```python
from build123d import *

# Parameters (mm, degrees)
BASE_EXTRUDE_DEPTH      = 1.5
BASE_EXTRUDE_DEPTH_BACK = 1.5
SKETCH1_R               = 2


with BuildPart() as part:
    # Sketch1 → Base-Extrude (new, two sides: drawn at the far end of the back side and taken through both)
    with BuildSketch(Plane.XY.offset(-BASE_EXTRUDE_DEPTH_BACK)):
        with BuildLine():
            Line((-14.708808387, -54.894020219), (-16.435009364, -61.336289969))
            ThreePointArc((-16.435009364, -61.336289969), (0, 63.5), (16.435009364, -61.336289969))
            Line((16.435009364, -61.336289969), (14.708808387, -54.894020219))
            ThreePointArc((14.708808387, -54.894020219), (17.560433321, -49.007812256), (23.796756449, -50.979482305))
            ThreePointArc((23.796756449, -50.979482305), (25.28518113, -52.085758206), (27.1261898, -51.862282302))
            ThreePointArc((27.1261898, -51.862282302), (0, 54.2), (-27.1261898, -51.862282302))
            ThreePointArc((-27.1261898, -51.862282302), (-25.28518113, -52.085758206), (-23.796756449, -50.979482305))
            ThreePointArc((-23.796756449, -50.979482305), (-17.560433321, -49.007812256), (-14.708808387, -54.894020219))
        make_face()
        with Locations((-19.733291854, -54.327131275)):
            Circle(SKETCH1_R, mode=Mode.SUBTRACT)
        with Locations(Location((19.733291854, -54.327131275, 0), (0, 0, 180))):
            Circle(SKETCH1_R, mode=Mode.SUBTRACT)
    extrude(amount=BASE_EXTRUDE_DEPTH + BASE_EXTRUDE_DEPTH_BACK)


solid = part.part
```
Source: CAD feature listing. Evaluate the final solid. Frame: model axes, mm. A direction names the side the tool comes from. Coordinates: 2 decimals unless noted, no trailing zeros. Order: outer loops, then holes, each group sorted by start corner. A loop starts at its lowest first (then second) coordinate and runs counter-clockwise, first axis right, second up. Notation, with made-up numbers: M -29.5,68.25 L -10.5,68.25 A22 cw -10.5,87.25 Z; hole C -12.75,81.5 d3. An arc over 180 degrees is marked long. Write each question's results on one line, items separated by ' | '. Start each with the question number.
1) Section query D-D (x = 0). Return the cut outline in (y, z), plus the area to 3 significant figures.
2) Section query C-C (x = -40). Return the cut outline in (y, z).
3) Section query B-B (z = -0.95). Return the cut outline in (x, y) (3 decimals).
4) Contact query for flat-ended pins moving along their axis: pin 1 Ø1.5 at (x, z) = (-36.5, 1) entering from -Y; pin 2 Ø1.5 at (y, z) = (-0.5, 0) entering from +X; pin 3 Ø5 at (x, y) = (19.73, -54.33) entering from +Z. Output: stop coordinate, or through.
5) Draft query along Y for faces 4 (the face through (-15.56, -58.07, -0.02)), 5 (the face through (-25.311, -52.092, -0.021)), 6 (the face through (-2.56, 63.45, -0.02)). Return one class per face: released by +Y, released by -Y, zero draft, split by the parting line, or undercut.
6) Section query A-A (y = -2.3). Return the cut outline in (x, z), plus the area to 4 significant figures.
7) Access query for faces 1 (the face through (19, 52, -1.5)), 2 (the face through (15.584, -58.16, -0.021)), 3 (the face through (25.26, -52.08, -0.02)). Directions: +Z, -Z, +X, -X, +Y, -Y. A direction counts if a zero-diameter tool reaches every point of the face in a straight line with its end or side. Return the directions, or none.
8) Line query: line 1 (X direction, y = -42, z = -1); line 2 (X direction, y = -2.3, z = 0.2); line 3 (Y direction, x = 26.5, z = 0.55). Output: solid intervals per line, ascending. Write a range as from..to.
Answers:
1) outline: M 54.2,-1.5 L 63.5,-1.5 L 63.5,1.5 L 54.2,1.5 Z | area: 27.9 mm^2
2) outline: M -49.32,-1.5 L -42.2,-1.5 L -42.2,1.5 L -49.32,1.5 Z; M 37.6,-1.5 L 49.32,-1.5 L 49.32,1.5 L 37.6,1.5 Z
3) outline: M -27.126,-51.862 A56.5 cw long 27.126,-51.862 A2.5 cw 23.797,-50.979 A5 ccw 14.709,-54.894 L 16.435,-61.336 A63.5 ccw long -16.435,-61.336 L -14.709,-54.894 A5 ccw -23.797,-50.979 A2.5 cw Z; hole C -19.733,-54.327 d4; hole C 19.733,-54.327 d4
4) pin 1: stops at y = -52.48 | pin 2: stops at x = 63.5 | pin 3: stops at z = 1.5
5) face 4: released by -Y | face 5: undercut | face 6: split by the parting line
6) outline: M -63.46,-1.5 L -56.5,-1.5 L -56.5,1.5 L -63.46,1.5 Z; M 56.5,-1.5 L 63.46,-1.5 L 63.46,1.5 L 56.5,1.5 Z | area: 41.75 mm^2
7) face 1: -Z, +X, -X, +Y, -Y | face 2: +Z, -Z, -Y | face 3: +Z, -Z
8) line 1: x = -47.63..-40.2, 40.2..47.63 | line 2: x = -63.46..-56.5, 56.5..63.46 | line 3: y = -57.71..-52.1, 47.6..57.71
